```python
from build123d import *

# Parameters (mm, degrees)
HEXAGONSOCKET_DEPTH = 1.1
HEADFILLET_R        = 0.25
CHAMFER_2_SIZE      = 0.55
SKETCH4_W           = 5
SKETCH4_H           = 5


with BuildPart() as part:
    # Sketch1 → Base (revolve)
    with BuildSketch(Plane.XY, mode=Mode.PRIVATE) as base_sk:
        Polygon((0, 0), (0, 6.72), (3.72, 3), (10, 3), (10, 0), align=None)
    revolve(base_sk.sketch.rotate(Axis((-0.587069181, 0, 0), (1, 0, 0)), 90), axis=Axis((-0.587069181, 0, 0), (1, 0, 0)))

    # Sketch2 → HexagonSocket (cut)
    with BuildSketch(Plane(origin=(0, 0, 0), x_dir=(0, 0, -1), z_dir=(1, 0, 0))):
        Polygon((2.309401077, 0), (1.154700538, 2), (-1.154700538, 2), (-2.309401077, 0), (-1.154700538, -2), (1.154700538, -2), align=None)
    extrude(amount=HEXAGONSOCKET_DEPTH, mode=Mode.SUBTRACT)

    # Sketch3 → Cut-Revolve1 (revolve, cut)
    with BuildSketch(Plane.XY, mode=Mode.PRIVATE) as cut_revolve1_sk:
        Polygon((1.1, 2), (2.254700538, 0), (1.1, 0), align=None)
    revolve(cut_revolve1_sk.sketch.rotate(Axis((-0.439109555, 0, 0), (1, 0, 0)), 90), axis=Axis((-0.439109555, 0, 0), (1, 0, 0)), mode=Mode.SUBTRACT)

    # HeadFillet
    headfillet_edges = [part.edges().sort_by_distance(p)[0] for p in [
        (3.72, 0, -3),
    ]]
    fillet(headfillet_edges, radius=HEADFILLET_R)

    # Chamfer 2
    chamfer_2_edges = [part.edges().sort_by_distance(p)[0] for p in [
        (10, 0, -3),
    ]]
    chamfer(chamfer_2_edges, length=CHAMFER_2_SIZE)

    # Sketch4 → Cut-Revolve2 (revolve, cut)
    with BuildSketch(Plane(origin=(0, 0, 0), x_dir=(1, 0, 0), z_dir=(0, 1, 0)), mode=Mode.PRIVATE) as cut_revolve2_sk:
        with Locations((0.5, 8.17)):
            Rectangle(SKETCH4_W, SKETCH4_H)
    revolve(cut_revolve2_sk.sketch.rotate(Axis((11.853138686, 0, 0), (-1, 0, 0)), 180), axis=Axis((11.853138686, 0, 0), (-1, 0, 0)), mode=Mode.SUBTRACT)


solid = part.part
```
Build history of the part. All positions in model axes, mm. A direction names the side the tool comes from. Give positions to 0.01 mm unless a question says otherwise; leave off trailing zeros. Loops run counter-clockwise (first coordinate to the right, second up) from the corner with the lowest first, then second, coordinate; pieces in that order, holes last.
Item 1: Which spindle directions (+Z, -Z, +X, -X, +Y, -Y) get a long thin tool onto all of the face, cutting with end or side? Do faces 1 (the face through (0.54, -0.99, 1.74)), 2 (the face through (0, -0.08, -2.44)). Say none if no direction does.
Answers follow:
face 1: -X
face 2: +Z, -Z, -X, +Y, -Y
Item 2: Pull direction Y, two halves, no side cores. Call faces 3 (the face through (10, 0, 0)), 4 (the face through (6.68, 1.15, 2.77)), 5 (the face through (2.07, 0.31, -0.07)): released by +Y, released by -Y, zero draft, split by the parting line, or undercut.
Answers follow:
face 3: zero draft
face 4: split by the parting line
face 5: undercut
Item 3: Flat gauge pins, fed straight in: pin 1 (5 mm diameter, centred on y = -3, z = 2, fed in from +X); pin 2 (0.6 mm diameter, centred on x = 0.5, z = -0.5, fed in from +Y); pin 3 (0.6 mm diameter, centred on x = 0.5, z = -0.5, fed in from -Y); pin 4 (4 mm diameter, centred on x = 5, z = 0.5, fed in from -Y). Where does each tip first touch, or does it go through?
Answers follow:
pin 1: stops at x = 10
pin 2: stops at y = 5.67
pin 3: stops at y = -5.67
pin 4: stops at y = -3.7
Item 4: Drill centre lines: line 1 (Z direction, x = 4, y = -0.5); line 2 (Y direction, x = 3.5, z = 2.5); line 3 (Z direction, x = 9, y = -2.75). Where is each one in solid material? Low to high.
Answers follow:
line 1: z = -2.96 to 2.96
line 2: y = -2.03 to 2.03
line 3: z = -1.2 to 1.2
Item 5: Slice it at A-A, the plane x = 7. List the corners of the cut face in (y, z), and give its area (3 significant figures).
Answers follow:
outline: circle Ø6 at (0, 0)
area: 28.3 mm2
